Build history of the part. All positions in model axes, mm. Give positions to 0.01 mm unless a question says otherwise; leave off trailing zeros. One line per item, written item: value.
```python
from build123d import *

# Parameters (mm, degrees)
SKETCH_1_R      = 2.1
SKETCH_1_R_2    = 3.4
EXTRUDE_1_DEPTH = 940


with BuildPart() as part:
    # 草图1 → 拉伸1 (new body)
    with BuildSketch(Plane(origin=(0, 0, 0), x_dir=(1, 0, 0), z_dir=(0, 1, 0))):
        with BuildLine():
            Line((6.75, -28), (11, -28))
            Line((11, -28), (11, -30))
            Line((11, -30), (2, -30))
            ThreePointArc((2, -30), (0.585786438, -29.414213562), (0, -28))
            Line((0, -28), (0, -19))
            Line((0, -19), (2, -19))
            Line((2, -19), (2, -23.25))
            Line((2, -23.25), (5.335785999, -23.25))
            Line((5.335785999, -23.25), (9, -19.585785999))
            Line((9, -19.585785999), (9, -10.414214001))
            Line((9, -10.414214001), (5.335785999, -6.75))
            Line((5.335785999, -6.75), (2, -6.75))
            Line((2, -6.75), (2, -11))
            Line((2, -11), (0, -11))
            Line((0, -11), (0, -2))
            ThreePointArc((0, -2), (0.585786438, -0.585786438), (2, 0))
            Line((2, 0), (11, 0))
            Line((11, 0), (11, -2))
            Line((11, -2), (6.75, -2))
            Line((6.75, -2), (6.75, -5.335785999))
            Line((6.75, -5.335785999), (10.414214001, -9))
            Line((10.414214001, -9), (19.585785999, -9))
            Line((19.585785999, -9), (23.25, -5.335785999))
            Line((23.25, -5.335785999), (23.25, -2))
            Line((23.25, -2), (19, -2))
            Line((19, -2), (19, 0))
            Line((19, 0), (28, 0))
            ThreePointArc((28, 0), (29.414213562, -0.585786438), (30, -2))
            Line((30, -2), (30, -11))
            Line((30, -11), (28, -11))
            Line((28, -11), (28, -6.75))
            Line((28, -6.75), (24.664214001, -6.75))
            Line((24.664214001, -6.75), (21, -10.414214001))
            Line((21, -10.414214001), (21, -19.585785999))
            Line((21, -19.585785999), (24.664214001, -23.25))
            Line((24.664214001, -23.25), (28, -23.25))
            Line((28, -23.25), (28, -19))
            Line((28, -19), (30, -19))
            Line((30, -19), (30, -28))
            ThreePointArc((30, -28), (29.414213562, -29.414213562), (28, -30))
            Line((28, -30), (19, -30))
            Line((19, -30), (19, -28))
            Line((19, -28), (23.25, -28))
            Line((23.25, -28), (23.25, -24.664214001))
            Line((23.25, -24.664214001), (19.585785999, -21))
            Line((19.585785999, -21), (10.414214001, -21))
            Line((10.414214001, -21), (6.75, -24.664214001))
            Line((6.75, -24.664214001), (6.75, -28))
        make_face()
        with Locations(Location((3.375, -26.625, 0), (0, 0, 90))):
            Circle(SKETCH_1_R, mode=Mode.SUBTRACT)
        with Locations(Location((26.625, -26.625, 0), (0, 0, 90))):
            Circle(SKETCH_1_R, mode=Mode.SUBTRACT)
        with Locations(Location((15, -15, 0), (0, 0, 90))):
            Circle(SKETCH_1_R_2, mode=Mode.SUBTRACT)
        with Locations(Location((3.375, -3.375, 0), (0, 0, 90))):
            Circle(SKETCH_1_R, mode=Mode.SUBTRACT)
        with Locations(Location((26.625, -3.375, 0), (0, 0, 90))):
            Circle(SKETCH_1_R, mode=Mode.SUBTRACT)
    extrude(amount=EXTRUDE_1_DEPTH)


solid = part.part
```
(1) Slice it at A-A, the plane y = 315. Count the separate pieces of the cut face and the enclosed holes in it, and give its area (3 significant figures).
Completed:
separate pieces: 1
enclosed holes: 5
area: 333 mm²
(2) Pin check, flat tips, straight feed: P1, Ø1.6, axis at y = 511, z = 29, coming from the -X side; P2, Ø1.6, axis at y = 382, z = 29, coming from the +X side; P3, Ø4, axis at x = 15, z = 15, coming from the -Y side; P4, Ø1.6, axis at y = 438.5, z = 0.5, coming from the +X side. Stop position of each tip, or through.
Completed:
P1: x = 0.01
P2: x = 29.99
P3: through
P4: x = 29.87
(3) Drill centre lines: line 1 (X direction, y = 812.5, z = 19.25); line 2 (X direction, y = 304.5, z = 3); line 3 (Z direction, x = 15, y = 437.5). Where is each one in solid material? Low to high.
Completed:
line 1: 0 to 2, 9 to 21, 28 to 30
line 2: 0 to 1.31, 5.44 to 6.75, 23.25 to 24.56, 28.69 to 30
line 3: 9 to 11.6, 18.4 to 21
